Geometry check sheet. Reference: the model listing, model coordinates, mm. Round coordinates to 2 decimals unless told otherwise and drop trailing zeros. Order: outer loops, then holes, each group sorted by start corner. A loop starts at its lowest first (then second) coordinate and runs counter-clockwise, first axis right, second up.
(1) Cross-section at A-A on y = 0. Enter the section's corners in (x, z), and give its area (3 significant figures).
(2) Cross-section at B-B on x = -21. Enter the section's corners in (y, z).
(3) Cross-section at D-D on x = 21.5. Enter the section's corners in (y, z).
(4) Cross-section at C-C on z = -0.95. Enter the section's corners in (x, y), and give its area (3 significant figures).
(5) Draft check along X on faces 1 (the face through (0, 6, 0)), 2 (the face through (-18.854, 0.676, -0.021)), 3 (the face through (25, 0, 0)). Enter one of: pulls with the +X half, pulls with the -X half, needs draft (parallel to the pull), parting line crosses it, or undercut.
(6) Thickness scan on L1, parallel to Y at x = 21, z = -0.7; L2, parallel to X at y = 1, z = 1.05; L3, parallel to X at y = -0.25, z = 0.55. Record the ranges inside material, lowest first.
from build123d import *

# Parameters (mm, degrees)
SKETCH_1_W      = 50
SKETCH_1_H      = 12
SKETCH_1_R      = 2.25
EXTRUDE_1_DEPTH = 1.5


with BuildPart() as part:
    # 草图1 → 凸台-拉伸1 (new, symmetric)
    with BuildSketch(Plane.XY):
        Rectangle(SKETCH_1_W, SKETCH_1_H)
        with Locations((-21, 0)):
            Circle(SKETCH_1_R, mode=Mode.SUBTRACT)
        with Locations((21, 0)):
            Circle(SKETCH_1_R, mode=Mode.SUBTRACT)
    extrude(amount=EXTRUDE_1_DEPTH, both=True)


solid = part.part
Found:
1. outline: (-25, -1.5) - (-23.25, -1.5) - (-23.25, 1.5) - (-25, 1.5) - close; (-18.75, -1.5) - (18.75, -1.5) - (18.75, 1.5) - (-18.75, 1.5) - close; (23.25, -1.5) - (25, -1.5) - (25, 1.5) - (23.25, 1.5) - close
1. area: 123 mm2
2. outline: (-6, -1.5) - (-2.25, -1.5) - (-2.25, 1.5) - (-6, 1.5) - close; (2.25, -1.5) - (6, -1.5) - (6, 1.5) - (2.25, 1.5) - close
3. outline: (-6, -1.5) - (-2.19, -1.5) - (-2.19, 1.5) - (-6, 1.5) - close; (2.19, -1.5) - (6, -1.5) - (6, 1.5) - (2.19, 1.5) - close
4. outline: (-25, -6) - (25, -6) - (25, 6) - (-25, 6) - close; hole circle Ø4.5 at (-21, 0); hole circle Ø4.5 at (21, 0)
4. area: 568 mm2
5. face 1: needs draft
5. face 2: undercut
5. face 3: pulls with the +X half
6. L1: y = -6 to -2.25, 2.25 to 6
6. L2: x = -25 to -23.02, -18.98 to 18.98, 23.02 to 25
6. L3: x = -25 to -23.24, -18.76 to 18.76, 23.24 to 25
